```python
from build123d import *

# Parameters (mm, degrees)
SKETCH_1_R      = 6.5
EXTRUDE_1_DEPTH = 6


with BuildPart() as part:
    # 草图1 → 凸台-拉伸1 (new body)
    with BuildSketch(Plane.XY):
        with BuildLine():
            Line((-42.5, 25), (42.5, 25))
            Line((42.5, 25), (42.5, -17))
            ThreePointArc((42.5, -17), (40.156854249, -22.656854249), (34.5, -25))
            Line((34.5, -25), (-34.5, -25))
            ThreePointArc((-34.5, -25), (-40.156854249, -22.656854249), (-42.5, -17))
            Line((-42.5, -17), (-42.5, 25))
        make_face()
        Circle(SKETCH_1_R, mode=Mode.SUBTRACT)
    extrude(amount=EXTRUDE_1_DEPTH)


solid = part.part
```
Can you work these out from the model? Positions are in its coordinate system, mm. Coordinates: 2 decimals unless noted, no trailing zeros. Write each loop counter-clockwise with the first axis right and the second up, starting at its lowest first coordinate (ties: lowest second). Pieces come first, ordered by that corner, then holes. Notation, with made-up numbers: (65, 70) - (101, 70) arc R12 ccw to (101, 93) - close; hole circle Ø6 at (62, -38). An arc over 180 degrees is marked (long way). Return JSON: item names as keys, results as strings.
Q1. If we section it at B-B (x = 0): Please give me the cut outline in (y, z).
Computed values:
{"outline": "(-25, 0) - (-6.5, 0) - (-6.5, 6) - (-25, 6) - close; (6.5, 0) - (25, 0) - (25, 6) - (6.5, 6) - close"}
Q2. I'm going to push a flat-ended pin straight in: pin 1 Ø2 at (x, y) = (14, 1) entering from -Z. Where does the tip first touch, or does it pass through?
Computed values:
{"pin 1": "stops at z = 0"}
Q3. If we section it at C-C (z = 4.4): Please give me the cut outline in (x, y), then the cut area to 3 significant figures.
Computed values:
{"outline": "(-42.5, -17) arc R8 ccw to (-34.5, -25) - (34.5, -25) arc R8 ccw to (42.5, -17) - (42.5, 25) - (-42.5, 25) - close; hole circle Ø13 at (0, 0)", "area": "4,090 mm2"}
Q4. If we section it at A-A (y = 0): Please give me the cut outline in (x, z).
Computed values:
{"outline": "(-42.5, 0) - (-6.5, 0) - (-6.5, 6) - (-42.5, 6) - close; (6.5, 0) - (42.5, 0) - (42.5, 6) - (6.5, 6) - close"}
Q5. Please list where these lines run through material, in increasing order: L1, parallel to Y at x = 0, z = 1.7; L2, parallel to X at y = -5, z = 4.65; L3, parallel to Y at x = -6, z = 4.95. Write a range as from..to.
Computed values:
{"L1": "y = -25..-6.5, 6.5..25", "L2": "x = -42.5..-4.15, 4.15..42.5", "L3": "y = -25..-2.5, 2.5..25"}
Q6. Thinking about a two-plate mould opening in X: for faces 1 (the cylindrical face through (-40.094, -22.719, 2.958)), 2 (the cylindrical face through (-5.158, -3.955, 2.958)), 3 (the flat face through (42.5, 4, 3)), which applies, +X half, -X half, draft (parallel to the pull), parting line (faces both ways), or undercut?
Computed values:
{"face 1": "-X half", "face 2": "undercut", "face 3": "+X half"}
